Verification items for the finished model (mm, model axes). Face numbers are marked on the shaded views. Round coordinates to 2 decimals unless told otherwise and drop trailing zeros. Order: outer loops, then holes, each group sorted by start corner. A loop starts at its lowest first (then second) coordinate and runs counter-clockwise, first axis right, second up. Notation, with made-up numbers: M 78.25,76 L 113.25,76 A36 cw 113.25,112 Z; hole C 12.5,54 d9. An arc over 180 degrees is marked long. Use one line per item in the form item = value. Start each with the question number.
Item 1: Thickness scan on probe 1 along X at (y, z) = (0, 1.05); probe 2 along Y at (x, z) = (-7.5, 1.15); probe 3 along X at (y, z) = (-2.75, 3.95) (3 decimals). Record the ranges inside material, lowest first. Write a range as [from, to].
Item 2: Cross-section at A-A on x = -7.5. Enter the section's corners in (y, z), then the cut area to 3 significant figures.
Item 3: Go/stop test with a flat-tipped pin: pin 1 Ø9 at (x, y) = (7.5, 0) entering from +Z. Record where the tip stops, or that it passes through.
Item 4: Release check for a two-part mould opening along Y. For the marked faces 1, 2 and 3 record: +Y half, -Y half, draft (parallel to the pull), parting line (faces both ways), or undercut.
Item 5: Cross-section at D-D on y = -2. Count the separate pieces of the cut face and the enclosed holes in it, then the cut area to 3 significant figures.
Item 6: Cross-section at B-B on y = 0. Enter the section's corners in (x, z).
Item 7: Cross-section at C-C on z = 2. Enter the section's corners in (x, y), then the cut area to 3 significant figures.
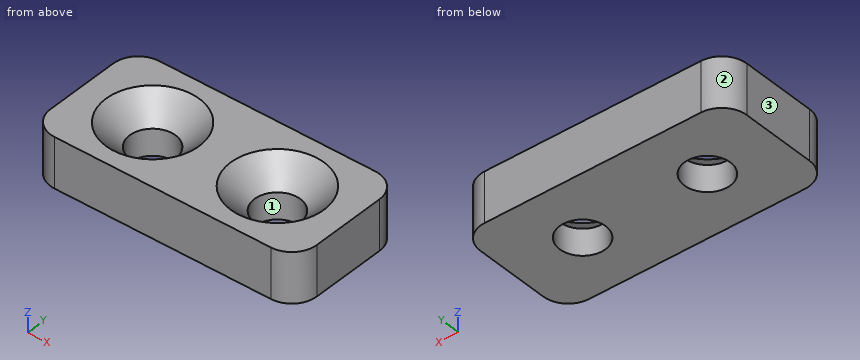
from build123d import *

# Parameters (mm, degrees)
SKETCH1_W                                            = 32
SKETCH1_H                                            = 15
BOSS_EXTRUDE1_DEPTH                                  = 6
CSK_FOR_M5_SLOTTED_RAISED_CTSK_HEAD_WOOD_D           = 5.5
CSK_FOR_M5_SLOTTED_RAISED_CTSK_HEAD_WOOD_DEPTH       = 12.4
CSK_FOR_M5_SLOTTED_RAISED_CTSK_HEAD_WOOD_CSINK_D     = 11.2
CSK_FOR_M5_SLOTTED_RAISED_CTSK_HEAD_WOOD_CSINK_ANGLE = 90
CSK_FOR_M5_SLOTTED_RAISED_CTSK_HEAD_WOOD_TIP         = 1.652366702
FILLET1_R                                            = 3


with BuildPart() as part:
    # Sketch1 → Boss-Extrude1 (new body)
    with BuildSketch(Plane.XY):
        Rectangle(SKETCH1_W, SKETCH1_H)
    extrude(amount=BOSS_EXTRUDE1_DEPTH)

    # CSK for M5 Slotted raised CTSK head wood screws1
    with Locations(Plane.XY.offset(6)):
        with Locations((7.5, 0), (60, 0), (-60, 0), (-7.5, 0)):
            CounterSinkHole(CSK_FOR_M5_SLOTTED_RAISED_CTSK_HEAD_WOOD_D / 2, CSK_FOR_M5_SLOTTED_RAISED_CTSK_HEAD_WOOD_CSINK_D / 2, depth=CSK_FOR_M5_SLOTTED_RAISED_CTSK_HEAD_WOOD_DEPTH, counter_sink_angle=CSK_FOR_M5_SLOTTED_RAISED_CTSK_HEAD_WOOD_CSINK_ANGLE)
            with Locations((0, 0, -(CSK_FOR_M5_SLOTTED_RAISED_CTSK_HEAD_WOOD_DEPTH + CSK_FOR_M5_SLOTTED_RAISED_CTSK_HEAD_WOOD_TIP / 2))):  # 118° drill point
                Cone(0, CSK_FOR_M5_SLOTTED_RAISED_CTSK_HEAD_WOOD_D / 2, CSK_FOR_M5_SLOTTED_RAISED_CTSK_HEAD_WOOD_TIP, mode=Mode.SUBTRACT)

    # Fillet1
    fillet1_edges = [part.edges().sort_by_distance(p)[0] for p in [
        (16, -7.5, 3),
        (-16, -7.5, 3),
        (-16, 7.5, 3),
        (16, 7.5, 3),
    ]]
    fillet(fillet1_edges, radius=FILLET1_R)


solid = part.part
Output values:
q1.probe_1 = [-16, -10.25], [-4.75, 4.75], [10.25, 16]
q1.probe_2 = [-7.5, -2.75], [2.75, 7.5]
q1.probe_3 = [-16, -9.745], [-5.255, 5.255], [9.745, 16]
q2.outline = M -7.5,0 L -2.75,0 L -2.75,3.15 L -5.6,6 L -7.5,6 Z; M 2.75,0 L 7.5,0 L 7.5,6 L 5.6,6 L 2.75,3.15 Z
q2.area = 48.9 mm2
q3.pin_1 = 4.9
q4.face_1 = undercut
q4.face_2 = +Y half
q4.face_3 = draft
q5.separate_pieces = 3
q5.enclosed_holes = 0
q5.area = 127 mm2
q6.outline = M -16,0 L -10.25,0 L -10.25,3.15 L -13.1,6 L -16,6 Z; M -4.75,0 L 4.75,0 L 4.75,3.15 L 1.9,6 L -1.9,6 L -4.75,3.15 Z; M 10.25,0 L 16,0 L 16,6 L 13.1,6 L 10.25,3.15 Z
q7.outline = M -16,-4.5 A3 ccw -13,-7.5 L 13,-7.5 A3 ccw 16,-4.5 L 16,4.5 A3 ccw 13,7.5 L -13,7.5 A3 ccw -16,4.5 Z; hole C -7.5,0 d5.5; hole C 7.5,0 d5.5
q7.area = 425 mm2
